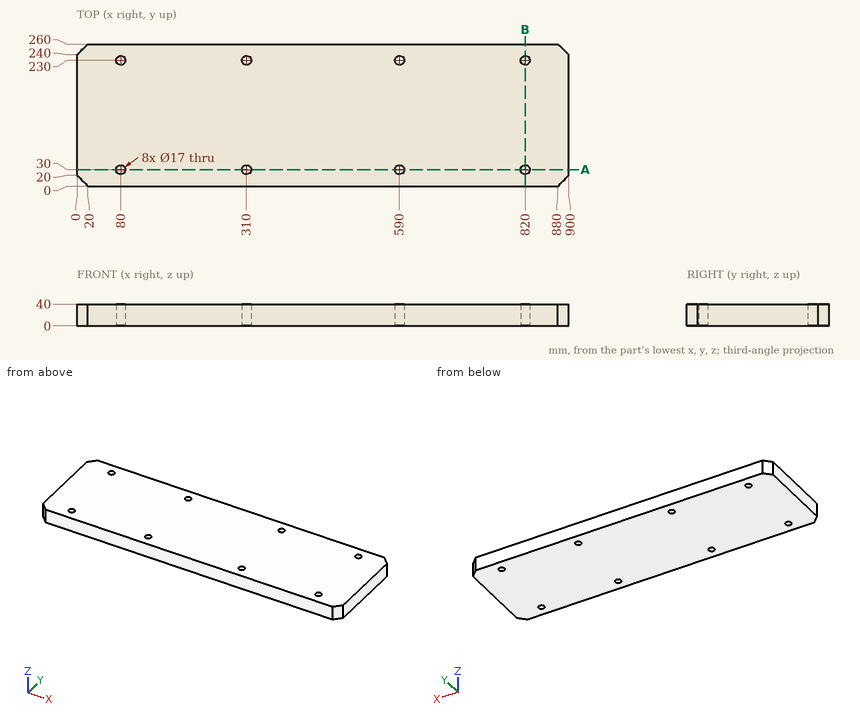
Geometry check sheet. Reference: drawing and pictorial views, mm from the part's lowest x, y, z. Round coordinates to 2 decimals unless told otherwise and drop trailing zeros. Loops run counter-clockwise (first coordinate to the right, second up) from the corner with the lowest first, then second, coordinate; pieces in that order, holes last. Notation, with made-up numbers: (1, 46) - (51, 46) arc R14 ccw to (51, 70) - close; hole circle Ø3 at (-11, -23). An arc over 180 degrees is marked (long way). Write item = value, one per line. Start each with the question number.
Q1. Section check B-B (x = 820). Record the boundary of the cut face in (y, z), plus the area to 3 significant figures.
Q2. Section check A-A (y = 30). Record the boundary of the cut face in (x, z), plus the area to 3 significant figures.
Q3. Thickness scan on L1, parallel to Y at x = 820, z = 17. Record the ranges inside material, lowest first.
Q4. Depth check by flat-ended pin: P1, Ø10, axis at x = 820, y = 230, coming from the +Z side. Enter the tip coordinate at first touch or a pass-through.
Derived:
q1.outline = (0, 0) - (21.5, 0) - (21.5, 40) - (0, 40) - close; (38.5, 0) - (221.5, 0) - (221.5, 40) - (38.5, 40) - close; (238.5, 0) - (260, 0) - (260, 40) - (238.5, 40) - close
q1.area = 9,040 mm^2
q2.outline = (0, 0) - (71.5, 0) - (71.5, 40) - (0, 40) - close; (88.5, 0) - (301.5, 0) - (301.5, 40) - (88.5, 40) - close; (318.5, 0) - (581.5, 0) - (581.5, 40) - (318.5, 40) - close; (598.5, 0) - (811.5, 0) - (811.5, 40) - (598.5, 40) - close; (828.5, 0) - (900, 0) - (900, 40) - (828.5, 40) - close
q2.area = 33,300 mm^2
q3.L1 = 0 to 21.5, 38.5 to 221.5, 238.5 to 260
q4.P1 = through
